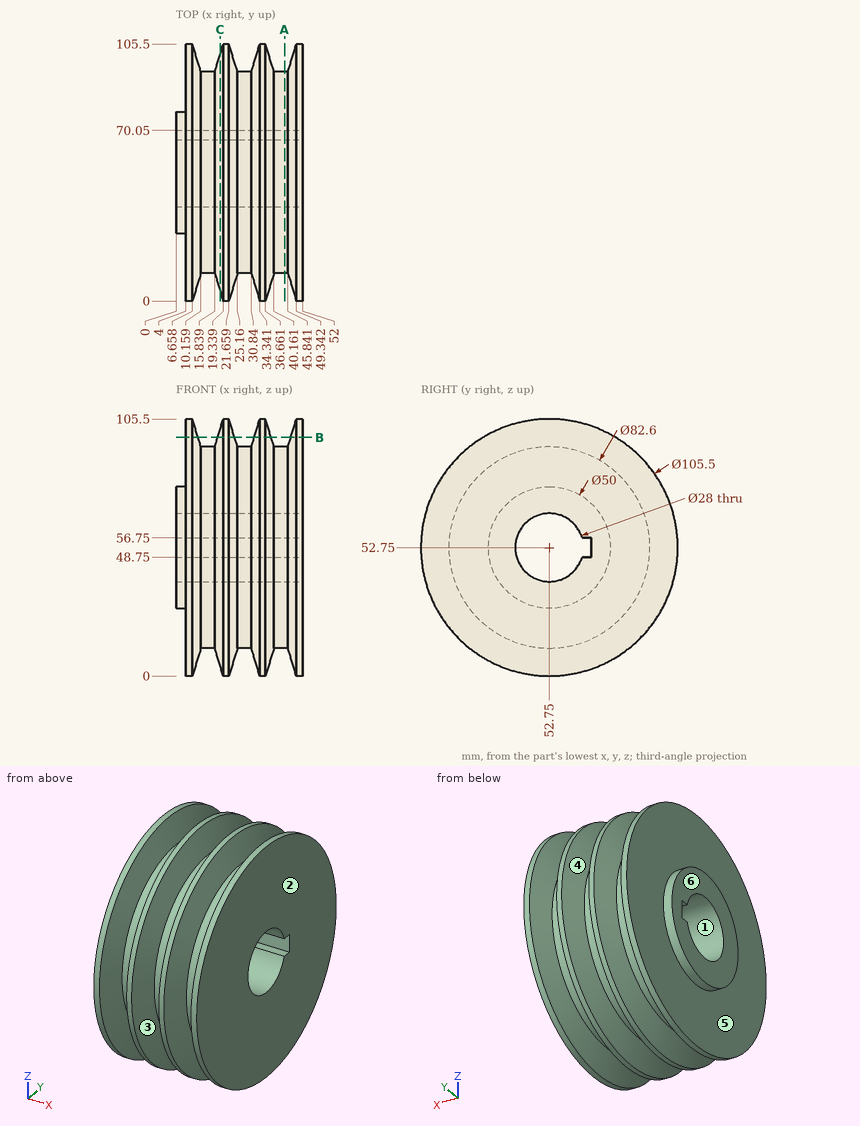
The figure shows three views and two pictorial views of one solid part (mm, origin at its lowest corner). Answer the questions. A direction names the side the tool comes from. Give positions to 0.01 mm unless a question says otherwise; leave off trailing zeros. Loops run counter-clockwise (first coordinate to the right, second up) from the corner with the lowest first, then second, coordinate; pieces in that order, holes last. Notation, with made-up numbers: M 27.5,-23 L 43.5,-23 A22 ccw 43.5,6 Z; hole C 63.5,55.5 d2. An arc over 180 degrees is marked long. Write each question's results on one line, items separated by ' | '.
1. A tool of negligible diameter and unlimited length cuts with its end or side. For the marked faces 4, 5 and 6, from which of +Z, -Z, +X, -X, +Y, -Y can it reach the whole face along a straight path? Write none if from no direction.
Values:
face 4: none | face 5: -X | face 6: +Z, -Z, -X, +Y, -Y
2. Section B-B on z = 98 is taken. State how many separate pieces and enclosed holes the cut face has, plus the area to 3 significant figures.
Values:
separate pieces: 4 | enclosed holes: 0 | area: 1,030 mm^2
3. Given pin 1 (4 mm diameter, centred on x = 38, z = 41.5, fed in from -Y); pin 2 (6.5 mm diameter, centred on x = 36.5, z = 54, fed in from -Y); pin 3 (3 mm diameter, centred on x = 19.5, y = 88.5, fed in from +Z), each flat-ended and moving along its own axis, determine where each tip first touches the part or whether it passes through.
Values:
pin 1: stops at y = 0.91 | pin 2: stops at y = 0 | pin 3: stops at z = 92.87
4. Section A-A on x = 44.5 is taken. Give the vertices of the cut face in (y, z), plus the area to 4 significant figures.
Values:
outline: C 52.75,52.75 d82.6; hole M 66.17,48.75 L 70.05,48.75 L 70.05,56.75 L 66.17,56.75 A14 ccw long Z | area: 4,715 mm^2
5. Straight lines are drawn through the part: line 1 (X direction, y = 98, z = 58); line 2 (X direction, y = 61.5, z = 6.5) (1 decimal); line 3 (Y direction, x = 14, z = 52.75). For each, find the intervals that lie inside material, in ascending order. Write a range as [from, to].
Values:
line 1: x = [4, 8.86], [17.14, 23.86], [32.14, 38.86], [47.14, 52] | line 2: x = [4, 8.4], [17.6, 23.4], [32.6, 38.4], [47.6, 52] | line 3: y = [11.45, 38.75], [70.05, 94.05]
6. The mould has two halves that part along Y. Classify the marked faces 1, 2 and 3: pulls with the +Y half, pulls with the -Y half, needs draft (parallel to the pull), parting line crosses it, or undercut.
Values:
face 1: undercut | face 2: needs draft | face 3: parting line crosses it
7. Section C-C on x = 18 is taken. Give the vertices of the cut face in (y, z).
Values:
outline: C 52.75,52.75 d96.74; hole M 66.17,48.75 L 70.05,48.75 L 70.05,56.75 L 66.17,56.75 A14 ccw long Z
